Read the model definition and answer for the solid it produces. Units are mm, in the model's axes. A direction names the side the tool comes from. Give positions to 0.01 mm unless a question says otherwise; leave off trailing zeros. Loops run counter-clockwise (first coordinate to the right, second up) from the corner with the lowest first, then second, coordinate; pieces in that order, holes last. Notation, with made-up numbers: (-2, 88.5) - (12, 88.5) arc R15 cw to (12, 108.5) - close; hole circle Ø3 at (56.5, 41.5). An arc over 180 degrees is marked (long way). Write item = value, one per line.
```python
from build123d import *

# Parameters (mm, degrees)
SKETCH_1_W          = 240
SKETCH_1_H          = 25
EXTRUDE_1_DEPTH     = 12
SKETCH_2_R          = 8
CUT_EXTRUDE_1_DEPTH = 2


with BuildPart() as part:
    # 草图1 → 凸台-拉伸1 (new body)
    with BuildSketch(Plane.XY):
        Rectangle(SKETCH_1_W, SKETCH_1_H)
    extrude(amount=EXTRUDE_1_DEPTH)

    # 草图2 → 切除-拉伸1 (cut)
    with BuildSketch(Plane.XY.offset(12)):
        with Locations((85, 0)):
            Circle(SKETCH_2_R)
        with Locations((-85, 0)):
            Circle(SKETCH_2_R)
    extrude(amount=-CUT_EXTRUDE_1_DEPTH, mode=Mode.SUBTRACT)


solid = part.part
```
1) A cutting plane is placed at B-B on y = 0. Determine the outline of the cut face in (x, z), then the cut area to 3 significant figures.
Output:
outline = (-120, 0) - (120, 0) - (120, 12) - (93, 12) - (93, 10) - (77, 10) - (77, 12) - (-77, 12) - (-77, 10) - (-93, 10) - (-93, 12) - (-120, 12) - close
area = 2,820 mm²
2) A tool of negligible diameter and unlimited length cuts with its end or side. For faces 1 (the face through (-2, 0, 12)), 2 (the face through (85, 0, 10)), from which of +Z, -Z, +X, -X, +Y, -Y can it reach the whole face along a straight path? Write none if from no direction.
Output:
face_1 = +Z, +X, -X, +Y, -Y
face_2 = +Z
3) A cutting plane is placed at A-A on x = 85. Determine the outline of the cut face in (y, z).
Output:
outline = (-12.5, 0) - (12.5, 0) - (12.5, 12) - (8, 12) - (8, 10) - (-8, 10) - (-8, 12) - (-12.5, 12) - close
4) Find the intervals of material crossed by probe 1 along Y at (x, z) = (-85, 11.3); probe 2 along Z at (x, y) = (91, 2.5), in increasing order.
Output:
probe_1 = -12.5 to -8, 8 to 12.5
probe_2 = 0 to 10
5) This flat-tipped pin is pushed along its axis until it touches: P1, Ø5, axis at x = -82.5, y = 3.5, coming from the +Z side. Where does it stop, or does it pass through?
Output:
P1 = 10
6) The mould has two halves that part along Y. Classify faces 3 (the face through (120, 0, 6)), 4 (the face through (-91.349, -4.868, 11.014)), 5 (the face through (-2, 12.5, 6)): pulls with the +Y half, pulls with the -Y half, needs draft (parallel to the pull), parting line crosses it, or undercut.
Output:
face_3 = needs draft
face_4 = undercut
face_5 = pulls with the +Y half
